```python
from build123d import *

# Parameters (mm, degrees)
BOSS_EXTRUDE1_DEPTH         = 5
BOSS_EXTRUDE2_DEPTH         = 6
BOSS_EXTRUDE3_DEPTH         = 6
SKETCH4_R                   = 8
CUT_EXTRUDE1_DEPTH          = 21
M8_TAPPED_HOLE1_D           = 6.8
M8_TAPPED_HOLE1_DEPTH       = 20
M8_TAPPED_HOLE1_CSINK_D     = 8.05
M8_TAPPED_HOLE1_CSINK_ANGLE = 90
M8_TAPPED_HOLE1_TIP         = 2.042926105
M6_TAPPED_HOLE1_D           = 5
M6_TAPPED_HOLE1_DEPTH       = 10
M6_TAPPED_HOLE1_CSINK_D     = 6.05
M6_TAPPED_HOLE1_CSINK_ANGLE = 90
M6_TAPPED_HOLE1_TIP         = 1.502151548


with BuildPart() as part:
    # Sketch1 → Boss-Extrude1 (new body)
    with BuildSketch(Plane.XY):
        with BuildLine():
            Line((-35, -12), (35, -12))
            ThreePointArc((35, -12), (38.535533906, -10.535533906), (40, -7))
            Line((40, -7), (40, 7))
            ThreePointArc((40, 7), (38.535533906, 10.535533906), (35, 12))
            Line((35, 12), (-35, 12))
            ThreePointArc((-35, 12), (-38.535533906, 10.535533906), (-40, 7))
            Line((-40, 7), (-40, -7))
            ThreePointArc((-40, -7), (-38.535533906, -10.535533906), (-35, -12))
        make_face()
    extrude(amount=BOSS_EXTRUDE1_DEPTH)

    # Sketch2 → Boss-Extrude2 (add, symmetric)
    with BuildSketch(Plane(origin=(0, 0, 0), x_dir=(1, 0, 0), z_dir=(0, 1, 0))):
        Polygon((-40, 0), (-22.5, 101), (22.5, 101), (40, 0), align=None)
    extrude(amount=BOSS_EXTRUDE2_DEPTH, both=True)

    # Sketch3 → Boss-Extrude3 (add)
    with BuildSketch(Plane(origin=(0, 6, 0), x_dir=(1, 0, 0), z_dir=(0, 1, 0))):
        with BuildLine():
            Line((-13, 14.5), (13, 14.5))
            ThreePointArc((13, 14.5), (16.535533906, 15.964466094), (18, 19.5))
            Line((18, 19.5), (18, 69.5))
            ThreePointArc((18, 69.5), (16.535533906, 73.035533906), (13, 74.5))
            Line((13, 74.5), (-13, 74.5))
            ThreePointArc((-13, 74.5), (-16.535533906, 73.035533906), (-18, 69.5))
            Line((-18, 69.5), (-18, 19.5))
            ThreePointArc((-18, 19.5), (-16.535533906, 15.964466094), (-13, 14.5))
        make_face()
    extrude(amount=BOSS_EXTRUDE3_DEPTH)

    # Sketch4 → Cut-Extrude1 (cut)
    with BuildSketch(Plane(origin=(0, 12, 0), x_dir=(1, 0, 0), z_dir=(0, 1, 0))):
        with Locations(Location((0, 54.5, 0), (0, 0, 270))):
            Circle(SKETCH4_R)
    extrude(amount=-CUT_EXTRUDE1_DEPTH, mode=Mode.SUBTRACT)

    # M8 Tapped Hole1
    with Locations(Plane(origin=(25, 0, 5), x_dir=(1, 0, 0), z_dir=(0, 0, 1))):
        with Locations((0, 0), (-50, 0)):
            CounterSinkHole(M8_TAPPED_HOLE1_D / 2, M8_TAPPED_HOLE1_CSINK_D / 2, depth=M8_TAPPED_HOLE1_DEPTH, counter_sink_angle=M8_TAPPED_HOLE1_CSINK_ANGLE)
            with Locations((0, 0, -(M8_TAPPED_HOLE1_DEPTH + M8_TAPPED_HOLE1_TIP / 2))):  # 118° drill point
                Cone(0, M8_TAPPED_HOLE1_D / 2, M8_TAPPED_HOLE1_TIP, mode=Mode.SUBTRACT)

    # M6 Tapped Hole1
    with Locations(Plane(origin=(14, 0, -101), x_dir=(-1, 0, 0), z_dir=(0, 0, -1))):
        with Locations((0, 0), (28, 0)):
            CounterSinkHole(M6_TAPPED_HOLE1_D / 2, M6_TAPPED_HOLE1_CSINK_D / 2, depth=M6_TAPPED_HOLE1_DEPTH, counter_sink_angle=M6_TAPPED_HOLE1_CSINK_ANGLE)
            with Locations((0, 0, -(M6_TAPPED_HOLE1_DEPTH + M6_TAPPED_HOLE1_TIP / 2))):  # 118° drill point
                Cone(0, M6_TAPPED_HOLE1_D / 2, M6_TAPPED_HOLE1_TIP, mode=Mode.SUBTRACT)


solid = part.part
```
CAD build for the part. Positions are in the model's coordinates, mm. A direction names the side the tool comes from. Round coordinates to 2 decimals unless told otherwise and drop trailing zeros. Order: outer loops, then holes, each group sorted by start corner. A loop starts at its lowest first (then second) coordinate and runs counter-clockwise, first axis right, second up.
Item 1: Saw through at A-A on x = 0. Write the cut outline in (y, z).
Item 2: Tool access for faces 5 (the face through (11.5, 0.1, -95.7)), 6 (the face through (0, 9, -74.5)), 7 (the face through (-1, -9, 0)): list every direction of +Z, -Z, +X, -X, +Y, -Y with a clear straight run to the whole face (end or side of a thin tool).
Item 3: Probe line 1 along Y through (x, z) = (-25, -6); line 2 along Y through (x, z) = (14, -98); line 3 along X through (y, z) = (0, -5.25). List the from-to ranges inside material, lowest first.
Item 4: Saw through at D-D on z = -38.5. Write the cut outline in (x, y).
Item 5: Mould opens along X. For faces 1 (the face through (0, 12, 2)), 2 (the face through (-18, 9, -45)), 3 (the face through (-4.868, 3.126, -60.849)), 4 (the face through (38, -11, 2)) say: pulls with the +X half, pulls with the -X half, needs draft (parallel to the pull), parting line crosses it, or undercut.
Item 6: Saw through at C-C on z = -61. Write the cut outline in (x, y), then the cut area to 3 significant figures.
Item 7: Saw through at B-B on y = 10.5. Write the cut outline in (x, z), then the cut area to 3 significant figures.
Item 8: Pin check, flat tips, straight feed: pin 1 (24 mm diameter, centred on x = 20, z = -27, fed in from -Y); pin 2 (1.8 mm diameter, centred on y = 10.5, z = -36, fed in from -X); pin 3 (6 mm diameter, centred on x = -14, y = 0, fed in from -Z) (3 decimals). Stop position of each tip, or through.
Reported:
1. outline: (-12, 0) - (-6, 0) - (-6, -46.5) - (12, -46.5) - (12, -14.5) - (6, -14.5) - (6, 0) - (12, 0) - (12, 5) - (-12, 5) - close; (-6, -101) - (6, -101) - (6, -74.5) - (12, -74.5) - (12, -62.5) - (-6, -62.5) - close
2. face 5: -Z
2. face 6: -Z, +X, -X, +Y
2. face 7: -Z, +X, -X, -Y
3. line 1: y = -6 to -3.4, 3.4 to 6
3. line 2: y = -6 to -2.5, 2.5 to 6
3. line 3: x = -39.09 to -28.4, -21.6 to 21.6, 28.4 to 39.09
4. outline: (-33.33, -6) - (33.33, -6) - (33.33, 6) - (18, 6) - (18, 12) - (-18, 12) - (-18, 6) - (-33.33, 6) - close
5. face 1: needs draft
5. face 2: pulls with the -X half
5. face 3: undercut
5. face 4: pulls with the +X half
6. outline: (-29.43, -6) - (-4.66, -6) - (-4.66, 12) - (-18, 12) - (-18, 6) - (-29.43, 6) - close; (4.66, -6) - (29.43, -6) - (29.43, 6) - (18, 6) - (18, 12) - (4.66, 12) - close
6. area: 754 mm2
7. outline: (-38.57, 0) - (38.57, 0) - (38.57, 5) - (-38.57, 5) - close; (-18, -69.5) arc R5 ccw to (-13, -74.5) - (13, -74.5) arc R5 ccw to (18, -69.5) - (18, -19.5) arc R5 ccw to (13, -14.5) - (-13, -14.5) arc R5 ccw to (-18, -19.5) - close; hole circle Ø16 at (0, -54.5)
7. area: 2,320 mm2
8. pin 1: stops at y = -6
8. pin 2: stops at x = -18
8. pin 3: stops at z = -100.975
